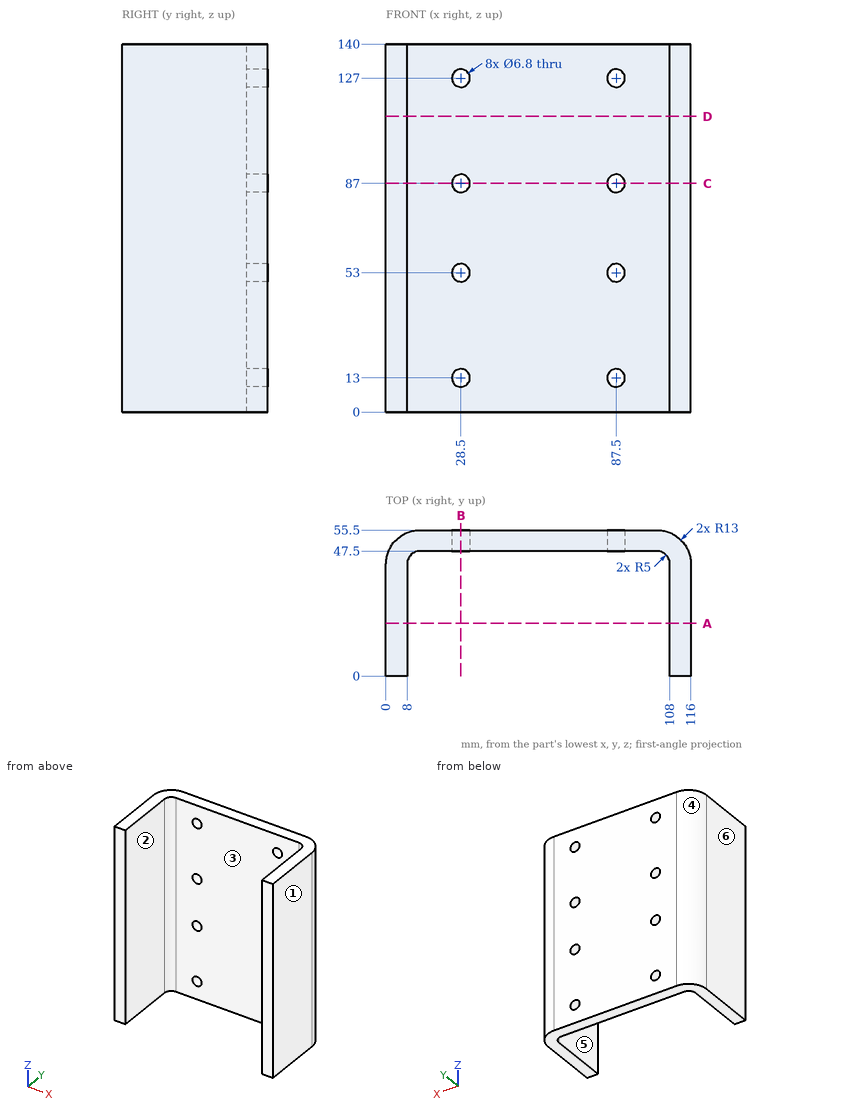
Can you work these out from the drawing? Everything is in mm from the part's minimum corner. A direction names the side the tool comes from. Give positions to 0.01 mm unless a question says otherwise; leave off trailing zeros. Order: outer loops, then holes, each group sorted by start corner. A loop starts at its lowest first (then second) coordinate and runs counter-clockwise, first axis right, second up. Notation, with made-up numbers: M 78,46 L 100,46 A4 ccw 100,53 Z; hole C 23,-23 d2. An arc over 180 degrees is marked long. Write item = value, one per line. Start each with the question number.
Q1. We'd pull the mould along X, two halves only. Please class the marked faces 1, 2, 3 and 4: pulls with the +X half, pulls with the -X half, needs draft (parallel to the pull), parting line crosses it, or undercut.
Q2. For the marked faces 5 and 6, which set-ups out of +Z, -Z, +X, -X, +Y, -Y let a thin tool reach every point of the face, with its end or its side?
Q3. Will these pins go through, and if not, where does the flat tip stop? pin 1 Ø5.5 at (x, z) = (87.5, 13) entering from -Y (3 decimals); pin 2 Ø3 at (x, z) = (11.5, 48.5) entering from -Y; pin 3 Ø8 at (x, z) = (87.5, 127) entering from -Y.
Q4. Suppose I cut it at C-C (z = 87). Write out the boundary of the cut face in (x, y), plus the area to 3 significant figures.
Q5. I need wall thicknesses on probe 1 along Z at (x, y) = (87.5, 53); probe 2 along X at (y, z) = (35.5, 9); probe 3 along X at (y, z) = (53, 87). Which ranges of each line are inside material? Lowest first, please. Write a range as [from, to].
Q6. Suppose I cut it at D-D (z = 112.5). Write out the boundary of the cut face in (x, y), plus the area to 3 significant figures.
Q7. Suppose I cut it at A-A (y = 20). Write out the boundary of the cut face in (x, z), plus the area to 3 significant figures.
Q8. Suppose I cut it at B-B (x = 28.5). Write out the boundary of the cut face in (y, z), plus the area to 3 significant figures.
Check result:
q1.face_1 = pulls with the +X half
q1.face_2 = undercut
q1.face_3 = undercut
q1.face_4 = pulls with the -X half
q2.face_5 = +Z, -Z, -Y
q2.face_6 = +Z, -Z, -X, +Y, -Y
q3.pin_1 = through
q3.pin_2 = 46.5
q3.pin_3 = 47.5
q4.outline = M 0,0 L 8,0 L 8,42.5 A5 cw 13,47.5 L 25.1,47.5 L 25.1,55.5 L 13,55.5 A13 ccw 0,42.5 Z; M 31.9,47.5 L 84.1,47.5 L 84.1,55.5 L 31.9,55.5 Z; M 90.9,47.5 L 103,47.5 A5 cw 108,42.5 L 108,0 L 116,0 L 116,42.5 A13 ccw 103,55.5 L 90.9,55.5 Z
q4.area = 1,520 mm2
q5.probe_1 = [0, 9.6], [16.4, 49.6], [56.4, 83.6], [90.4, 123.6], [130.4, 140]
q5.probe_2 = [0, 8], [108, 116]
q5.probe_3 = [5.34, 25.1], [31.9, 84.1], [90.9, 110.66]
q6.outline = M 0,0 L 8,0 L 8,42.5 A5 cw 13,47.5 L 103,47.5 A5 cw 108,42.5 L 108,0 L 116,0 L 116,42.5 A13 ccw 103,55.5 L 13,55.5 A13 ccw 0,42.5 Z
q6.area = 1,630 mm2
q7.outline = M 0,0 L 8,0 L 8,140 L 0,140 Z; M 108,0 L 116,0 L 116,140 L 108,140 Z
q7.area = 2,240 mm2
q8.outline = M 47.5,0 L 55.5,0 L 55.5,9.6 L 47.5,9.6 Z; M 47.5,16.4 L 55.5,16.4 L 55.5,49.6 L 47.5,49.6 Z; M 47.5,56.4 L 55.5,56.4 L 55.5,83.6 L 47.5,83.6 Z; M 47.5,90.4 L 55.5,90.4 L 55.5,123.6 L 47.5,123.6 Z; M 47.5,130.4 L 55.5,130.4 L 55.5,140 L 47.5,140 Z
q8.area = 902 mm2
